Verification items for the finished model (mm, model axes). A direction names the side the tool comes from. Round coordinates to 2 decimals unless told otherwise and drop trailing zeros. Write each loop counter-clockwise with the first axis right and the second up, starting at its lowest first coordinate (ties: lowest second). Pieces come first, ordered by that corner, then holes. Notation, with made-up numbers: (17.5, 62) - (27.5, 62) arc R25 cw to (27.5, 94) - close; hole circle Ø5 at (51, 27.5). An arc over 180 degrees is marked (long way). Write each question's results on one line, items separated by ' | '.
```python
from build123d import *

# Parameters (mm, degrees)
EXTRUDE_1_DEPTH     = 820
SKETCH_2_R          = 3.5
CUT_EXTRUDE_1_DEPTH = 820
CUT_EXTRUDE_2_DEPTH = 10


with BuildPart() as part:
    # 草图1 → 凸台-拉伸1 (new body)
    with BuildSketch(Plane.XY):
        with BuildLine():
            Line((0, 0), (28, 0))
            ThreePointArc((28, 0), (29.414213562, 0.585786438), (30, 2))
            Line((30, 2), (30, 41))
            ThreePointArc((30, 41), (31.464466094, 44.535533906), (35, 46))
            Line((35, 46), (931, 46))
            ThreePointArc((931, 46), (934.535533906, 44.535533906), (936, 41))
            Line((936, 41), (936, 2))
            ThreePointArc((936, 2), (936.585786438, 0.585786438), (938, 0))
            Line((938, 0), (966, 0))
            Line((966, 0), (966, -3))
            Line((966, -3), (938, -3))
            ThreePointArc((938, -3), (934.464466094, -1.535533906), (933, 2))
            Line((933, 2), (933, 41))
            ThreePointArc((933, 41), (932.414213562, 42.414213562), (931, 43))
            Line((931, 43), (35, 43))
            ThreePointArc((35, 43), (33.585786438, 42.414213562), (33, 41))
            Line((33, 41), (33, 2))
            ThreePointArc((33, 2), (31.535533906, -1.535533906), (28, -3))
            Line((28, -3), (0, -3))
            Line((0, -3), (0, 0))
        make_face()
    extrude(amount=EXTRUDE_1_DEPTH)

    # 草图2 → 切除-拉伸1 (cut)
    with BuildSketch(Plane(origin=(0, 46, 0), x_dir=(1, 0, 0), z_dir=(0, 1, 0))):
        with Locations(Location((53, -555, 0), (0, 0, 270))):
            Circle(SKETCH_2_R)
        with Locations(Location((53, -25, 0), (0, 0, 270))):
            Circle(SKETCH_2_R)
        with Locations(Location((913, -25, 0), (0, 0, 270))):
            Circle(SKETCH_2_R)
        with Locations(Location((913, -555, 0), (0, 0, 270))):
            Circle(SKETCH_2_R)
    extrude(amount=-CUT_EXTRUDE_1_DEPTH, mode=Mode.SUBTRACT)

    # 草图3 → 切除-拉伸2 (cut)
    with BuildSketch(Plane(origin=(0, 0, 0), x_dir=(1, 0, 0), z_dir=(0, 1, 0))):
        with BuildLine():
            Line((954.5, -82), (954.5, -88))
            ThreePointArc((954.5, -88), (950, -92.5), (945.5, -88))
            Line((945.5, -88), (945.5, -82))
            ThreePointArc((945.5, -82), (950, -77.5), (954.5, -82))
        make_face()
        with BuildLine():
            Line((954.5, -22), (954.5, -28))
            ThreePointArc((954.5, -28), (950, -32.5), (945.5, -28))
            Line((945.5, -28), (945.5, -22))
            ThreePointArc((945.5, -22), (950, -17.5), (954.5, -22))
        make_face()
        with BuildLine():
            Line((11.5, -82), (11.5, -88))
            ThreePointArc((11.5, -88), (16, -92.5), (20.5, -88))
            Line((20.5, -88), (20.5, -82))
            ThreePointArc((20.5, -82), (16, -77.5), (11.5, -82))
        make_face()
        with BuildLine():
            Line((11.5, -22), (11.5, -28))
            ThreePointArc((11.5, -28), (16, -32.5), (20.5, -28))
            Line((20.5, -28), (20.5, -22))
            ThreePointArc((20.5, -22), (16, -17.5), (11.5, -22))
        make_face()
        with BuildLine():
            Line((954.5, -787), (954.5, -793))
            ThreePointArc((954.5, -793), (950, -797.5), (945.5, -793))
            Line((945.5, -793), (945.5, -787))
            ThreePointArc((945.5, -787), (950, -782.5), (954.5, -787))
        make_face()
        with BuildLine():
            Line((11.5, -787), (11.5, -793))
            ThreePointArc((11.5, -793), (16, -797.5), (20.5, -793))
            Line((20.5, -793), (20.5, -787))
            ThreePointArc((20.5, -787), (16, -782.5), (11.5, -787))
        make_face()
    extrude(amount=-CUT_EXTRUDE_2_DEPTH, mode=Mode.SUBTRACT)


solid = part.part
```
(1) Thickness scan on L1, parallel to Z at x = 913, y = 43.85; L2, parallel to X at y = 32, z = 44.5; L3, parallel to X at y = 41.5, z = 261. Record the ranges inside material, lowest first.
Answer:
L1: 0 to 21.5, 28.5 to 551.5, 558.5 to 820 | L2: 30 to 33, 933 to 936 | L3: 30.03 to 33.06, 932.94 to 935.97
(2) Section check C-C (x = 300). Record the cut outline in (y, z), plus the area to 3 significant figures.
Answer:
outline: (43, 0) - (46, 0) - (46, 820) - (43, 820) - close | area: 2,460 mm2
(3) Section check A-A (y = 19). Record the cut outline in (x, z), plus the area to 3 significant figures.
Answer:
outline: (30, 0) - (33, 0) - (33, 820) - (30, 820) - close; (933, 0) - (936, 0) - (936, 820) - (933, 820) - close | area: 4,920 mm2
(4) Set-up check for faces 1 (the flat face through (14, -3, 404)), 2 (the flat face through (933, 21, 404)), 3 (the flat face through (952, 0, 404)), 4 (the flat face through (30, 21, 404)): record each of +Z, -Z, +X, -X, +Y, -Y from which the full face is reachable in a straight line by a thin tool's end or side.
Answer:
face 1: +Z, -Z, +X, -X, -Y | face 2: +Z, -Z, -Y | face 3: +Z, -Z, +X, +Y | face 4: +Z, -Z, -X, +Y
(5) Section check B-B (z = 391). Record the cut outline in (x, y), plus the area to 3 significant figures.
Answer:
outline: (0, -3) - (28, -3) arc R5 ccw to (33, 2) - (33, 41) arc R2 cw to (35, 43) - (931, 43) arc R2 cw to (933, 41) - (933, 2) arc R5 ccw to (938, -3) - (966, -3) - (966, 0) - (938, 0) arc R2 cw to (936, 2) - (936, 41) arc R5 ccw to (931, 46) - (35, 46) arc R5 ccw to (30, 41) - (30, 2) arc R2 cw to (28, 0) - (0, 0) - close | area: 3,160 mm2
(6) Go/stop test with flat-tipped pins: pin 1 Ø12 at (x, y) = (534, 34) entering from -Z; pin 2 Ø5 at (y, z) = (10, 557.5) entering from -X; pin 3 Ø2.5 at (y, z) = (-1, 23.5) entering from -X; pin 4 Ø3 at (y, z) = (26, 229) entering from +X. Record where each tip stops, or that it passes through.
Answer:
pin 1: through | pin 2: x = 30 | pin 3: x = 0 | pin 4: x = 936
